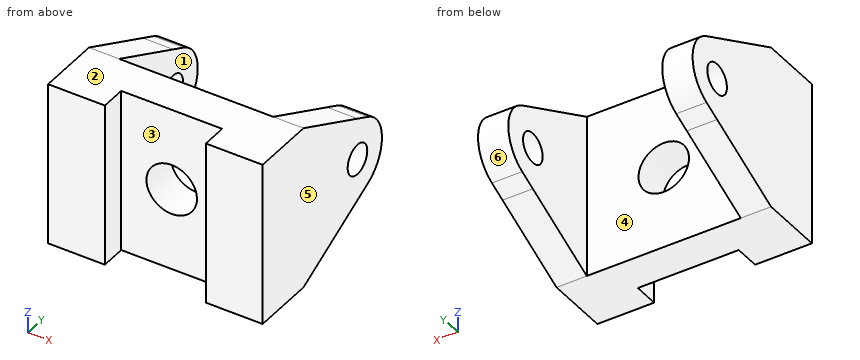
from build123d import *
from build123d.topology import SkipClean

# Parameters (mm, degrees)
BASE_BLOCK_DEPTH     = 32.5
CENTRE_HOLE_SKETCH_R = 10
CENTRE_HOLE_20_DEPTH = 65
LUG_A_BOSS_DEPTH     = 12
LUG_TRIM_CUT_DEPTH   = 102.080413533
LUG_B_BOSS_DEPTH     = 12
PIN_HOLE_SKETCH_R    = 6
PIN_HOLE_CUT_DEPTH   = 102.080413533
LUG_START            = -12
LUG_C_BOSS_DEPTH     = 12
LUG_RIB_A_SKETCH_W   = 61
LUG_RIB_A_SKETCH_H   = 4.481596486
LUG_RIB_A_DEPTH      = 13
LUG_RIB_B_SKETCH_W   = 61
LUG_RIB_B_SKETCH_H   = 4.481596486
LUG_RIB_B_DEPTH      = 13


with BuildPart() as part:
    # Base Profile Sketch → Base Block (new, symmetric)
    with BuildSketch(Plane.XY):
        Polygon((-42.5, 29), (-30.5, 29), (-30.5, -4), (30.5, -4), (30.5, 29), (42.5, 29), (42.5, -29), (20, -29), (20, -19), (-20, -19), (-20, -29), (-42.5, -29), align=None)
    extrude(amount=BASE_BLOCK_DEPTH, both=True)

    # Centre Hole Sketch → Centre Hole Ø20 (cut)
    with BuildSketch(Plane(origin=(0, -4, 0), x_dir=(1, 0, 0), z_dir=(0, 1, 0))):
        with Locations(Location((0, 0, 0), (0, 0, 270))):
            Circle(CENTRE_HOLE_SKETCH_R)
    extrude(amount=-CENTRE_HOLE_20_DEPTH, mode=Mode.SUBTRACT)

    # Lug A Sketch → Lug A Boss (add)
    with BuildSketch(Plane(origin=(42.5, 0, 0), x_dir=(0, 0, -1), z_dir=(1, 0, 0))):
        with BuildLine():
            ThreePointArc((13.519974515, 35.496944598), (0, 44), (-13.519974515, 35.496944598))
            ThreePointArc((-13.519974515, 35.496944598), (-14.625313975, 32.331694935), (-15, 29))
            Line((-15, 29), (-6, 29))
            ThreePointArc((-6, 29), (0, 35), (6, 29))
            Line((6, 29), (15, 29))
            ThreePointArc((15, 29), (14.625313975, 32.331694935), (13.519974515, 35.496944598))
        make_face()
        with BuildLine():
            Line((-6, 29), (-15, 29))
            ThreePointArc((-15, 29), (0, 14), (15, 29))
            Line((15, 29), (6, 29))
            ThreePointArc((6, 29), (0, 23), (-6, 29))
        make_face()
        with BuildLine():
            ThreePointArc((13.519974515, 35.496944598), (0, 44), (-13.519974515, 35.496944598))
            ThreePointArc((-13.519974515, 35.496944598), (-14.625313975, 32.331694935), (-15, 29))
            Line((-15, 29), (-6, 29))
            ThreePointArc((-6, 29), (0, 35), (6, 29))
            Line((6, 29), (15, 29))
            ThreePointArc((15, 29), (14.625313975, 32.331694935), (13.519974515, 35.496944598))
        make_face()
        with BuildLine():
            Line((-6, 29), (-15, 29))
            ThreePointArc((-15, 29), (0, 14), (15, 29))
            Line((15, 29), (6, 29))
            ThreePointArc((6, 29), (0, 23), (-6, 29))
        make_face()
        with BuildLine():
            Line((-16.642043204, 29), (-32.5, -4))
            Line((-32.5, -4), (32.5, -4))
            Line((32.5, -4), (16.642043204, 29))
            Line((16.642043204, 29), (15, 29))
            ThreePointArc((15, 29), (0, 14), (-15, 29))
            Line((-15, 29), (-16.642043204, 29))
        make_face()
        with BuildLine():
            Line((-13.519974515, 35.496944598), (-16.642043204, 29))
            Line((-16.642043204, 29), (-15, 29))
            ThreePointArc((-15, 29), (-14.625313975, 32.331694935), (-13.519974515, 35.496944598))
        make_face()
        with BuildLine():
            Line((15, 29), (16.642043204, 29))
            Line((16.642043204, 29), (13.519974515, 35.496944598))
            ThreePointArc((13.519974515, 35.496944598), (14.625313975, 32.331694935), (15, 29))
        make_face()
    extrude(amount=-LUG_A_BOSS_DEPTH)

    # Lug Trim Sketch → Lug Trim Cut (cut, through all)
    with BuildSketch(Plane(origin=(42.5, 0, 0), x_dir=(0, 0, -1), z_dir=(1, 0, 0))):
        Polygon((-32.5, -17), (-16.642043204, 29), (-32.5, 29), align=None)
        Polygon((32.5, -17), (16.642043204, 29), (32.5, 29), align=None)
    extrude(amount=-LUG_TRIM_CUT_DEPTH, mode=Mode.SUBTRACT)

    # Lug B Sketch → Lug B Boss (add)
    with BuildSketch(Plane(origin=(42.5, 0, 0), x_dir=(0, 0, -1), z_dir=(1, 0, 0))):
        Polygon((-16.642043204, 29), (-32.5, -4), (-32.5, -17), align=None)
        Polygon((32.5, -4), (32.5, -17), (16.642043204, 29), align=None)
    extrude(amount=-LUG_B_BOSS_DEPTH)

    # Pin Hole Sketch → Pin Hole Cut (cut, through all)
    with SkipClean():  # the faces are left unmerged after this step: merging them gives an invalid solid
        with BuildSketch(Plane(origin=(42.5, 0, 0), x_dir=(0, 0, -1), z_dir=(1, 0, 0))):
            with Locations(Location((0, 29, 0), (0, 0, 90))):
                Circle(PIN_HOLE_SKETCH_R)
        extrude(amount=-PIN_HOLE_CUT_DEPTH, mode=Mode.SUBTRACT)

    # Lug C Sketch → Lug C Boss (add)
    with SkipClean():  # the faces are left unmerged after this step: merging them gives an invalid solid
        with BuildSketch(Plane.ZY.offset(42.5).offset(LUG_START)):
            with BuildLine():
                ThreePointArc((13.519974515, 35.496944598), (0, 44), (-13.519974515, 35.496944598))
                ThreePointArc((-13.519974515, 35.496944598), (-14.625313975, 32.331694935), (-15, 29))
                Line((-15, 29), (-6, 29))
                ThreePointArc((-6, 29), (0, 35), (6, 29))
                Line((6, 29), (15, 29))
                ThreePointArc((15, 29), (14.625313975, 32.331694935), (13.519974515, 35.496944598))
            make_face()
            Polygon((-32.5, -4), (-16.642043204, 29), (-32.5, -17), align=None)
            Polygon((32.5, -17), (32.5, -4), (16.642043204, 29), align=None)
            with BuildLine():
                Line((-13.519974515, 35.496944598), (-16.642043204, 29))
                Line((-16.642043204, 29), (-15, 29))
                ThreePointArc((-15, 29), (-14.625313975, 32.331694935), (-13.519974515, 35.496944598))
            make_face()
            with BuildLine():
                Line((16.642043204, 29), (13.519974515, 35.496944598))
                ThreePointArc((13.519974515, 35.496944598), (14.625313975, 32.331694935), (15, 29))
                Line((15, 29), (16.642043204, 29))
            make_face()
        extrude(amount=LUG_C_BOSS_DEPTH)

    # Lug Rib A Sketch → Lug Rib A (add)
    with SkipClean():  # the faces are left unmerged after this step: merging them gives an invalid solid
        with BuildSketch(Plane(origin=(0, -4, 0), x_dir=(1, 0, 0), z_dir=(0, 1, 0))):
            with Locations((0, 30.259201757)):
                Rectangle(LUG_RIB_A_SKETCH_W, LUG_RIB_A_SKETCH_H)
        extrude(amount=-LUG_RIB_A_DEPTH)

    # Lug Rib B Sketch → Lug Rib B (add)
    with SkipClean():  # the faces are left unmerged after this step: merging them gives an invalid solid
        with BuildSketch(Plane(origin=(0, -4, 0), x_dir=(1, 0, 0), z_dir=(0, 1, 0))):
            with Locations((0, -30.259201757)):
                Rectangle(LUG_RIB_B_SKETCH_W, LUG_RIB_B_SKETCH_H)
        extrude(amount=-LUG_RIB_B_DEPTH)


solid = part.part
Source: CAD feature listing. Evaluate the final solid. Frame: model axes, mm. Face numbers are marked on the shaded views. A direction names the side the tool comes from. Give positions to 0.01 mm unless a question says otherwise; leave off trailing zeros. Write each loop counter-clockwise with the first axis right and the second up, starting at its lowest first coordinate (ties: lowest second). Pieces come first, ordered by that corner, then holes. Notation, with made-up numbers: M -8.5,68 L -4.5,68 A24 cw -4.5,80 Z; hole C 62,44 d2. An arc over 180 degrees is marked long. Return JSON: item names as keys, results as strings. Group by question number.
1) Set-up query: the marked faces 1, 2 and 3. Return all of +Z, -Z, +X, -X, +Y, -Y with unobstructed straight access to the full face (end or side cutting, diameter ignored); none if empty.
2) Cut plane A-A, the plane x = 0. Output: boundary loops of the cut face in (y, z), then the cut area to 3 significant figures.
3) Cut plane C-C, the plane y = -22. Output: boundary loops of the cut face in (x, z).
4) First-contact query: pin 1 Ø2 at (x, z) = (13, -23.5) entering from -Y; pin 2 Ø1 at (x, z) = (-9.5, 19.5) entering from +Y. Flat tips, straight axial feed; report the tip coordinate or a pass-through.
5) Draft query along X for the marked faces 4, 5 and 6. Return one class per face: released by +X, released by -X, zero draft, split by the parting line, or undercut.
6) Cut plane D-D, the plane z = 12. Output: boundary loops of the cut face in (x, y).
7) Ray query, L1, parallel to X at y = -23.5, z = 22.5; L2, parallel to X at y = -14, z = 0; L3, parallel to Y at x = -39.75, z = 0. Return the intervals inside material, ascending.
8) Cut plane B-B, the plane z = 0. Output: boundary loops of the cut face in (x, y).
Data:
{
 "1": {"face 1": "+Z, -Z, +Y", "face 2": "+Z, +X, -X, +Y, -Y", "face 3": "+Z, -Z, -Y"},
 "2": {"outline": "M -19,-32.5 L -4,-32.5 L -4,-10 L -19,-10 Z; M -19,10 L -4,10 L -4,32.5 L -19,32.5 Z", "area": "675 mm²"},
 "3": {"outline": "M -42.5,-32.5 L -20,-32.5 L -20,32.5 L -42.5,32.5 Z; M 20,-32.5 L 42.5,-32.5 L 42.5,32.5 L 20,32.5 Z"},
 "4": {"pin 1": "stops at y = -19", "pin 2": "stops at y = -4"},
 "5": {"face 4": "undercut", "face 5": "released by +X", "face 6": "zero draft"},
 "6": {"outline": "M -42.5,-29 L -20,-29 L -20,-19 L 20,-19 L 20,-29 L 42.5,-29 L 42.5,38 L 30.5,38 L 30.5,-4 L -30.5,-4 L -30.5,38 L -42.5,38 Z"},
 "7": {"L1": "x = -42.5 to -20, 20 to 42.5", "L2": "x = -42.5 to -10, 10 to 42.5", "L3": "y = -29 to 23, 35 to 44"},
 "8": {"outline": "M -42.5,-29 L -20,-29 L -20,-19 L -10,-19 L -10,-4 L -30.5,-4 L -30.5,23 L -42.5,23 Z; M -42.5,35 L -30.5,35 L -30.5,44 L -42.5,44 Z; M 10,-19 L 20,-19 L 20,-29 L 42.5,-29 L 42.5,23 L 30.5,23 L 30.5,-4 L 10,-4 Z; M 30.5,35 L 42.5,35 L 42.5,44 L 30.5,44 Z"}
}
